```python
from build123d import *

# Parameters (mm, degrees)
CUT_EXTRUDE_1_DEPTH = 4
CUT_EXTRUDE_START   = 31.9
SKETCH_3_R          = 15
SKETCH_3_R_2        = 14.3
CUT_EXTRUDE_2_DEPTH = 1.3


with BuildPart() as part:
    # 草图1 → 旋转1 (revolve)
    with BuildSketch(Plane.XY, mode=Mode.PRIVATE) as revolve_1_sk:
        Polygon((-360, 60), (360, 60), (360, 25), (370, 25), (370, 17.5), (454, 17.5), (454, 0), (-629, 0), (-629, 15), (-583, 15), (-583, 17.5), (-370, 17.5), (-370, 25), (-360, 25), align=None)
    revolve(revolve_1_sk.sketch.rotate(Axis((-629, 0, 0), (1, 0, 0)), 180), axis=Axis((-629, 0, 0), (1, 0, 0)))

    # 草图2 → 切除-拉伸1 (cut)
    with BuildSketch(Plane(origin=(0, 15, 0), x_dir=(1, 0, 0), z_dir=(0, 1, 0))):
        with BuildLine():
            Line((-629, 4), (-593, 4))
            ThreePointArc((-593, 4), (-589, 0), (-593, -4))
            Line((-593, -4), (-629, -4))
            Line((-629, -4), (-629, 4))
        make_face()
    extrude(amount=-CUT_EXTRUDE_1_DEPTH, mode=Mode.SUBTRACT)

    # 草图3 → 切除-拉伸2 (cut)
    with BuildSketch(Plane.ZY.offset(583).offset(CUT_EXTRUDE_START)):
        with Locations(Location((0, 0, 0), (0, 0, 270))):
            Circle(SKETCH_3_R)
        Circle(SKETCH_3_R_2, mode=Mode.SUBTRACT)
    extrude(amount=CUT_EXTRUDE_2_DEPTH, mode=Mode.SUBTRACT)


solid = part.part
```
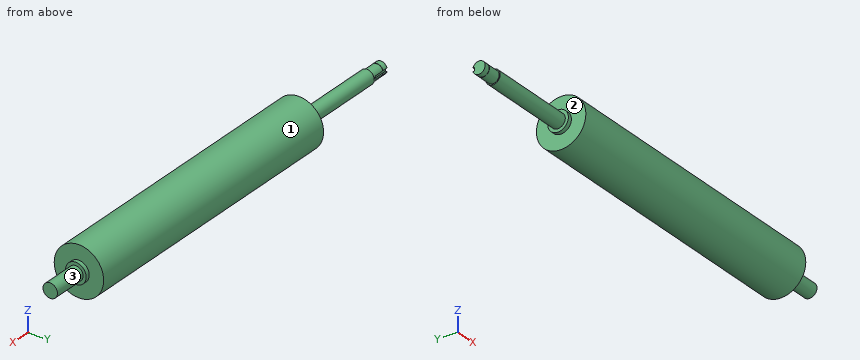
Check sheet for the modelled part. Datum: model origin and axes. Units: mm. Face numbers are marked on the shaded views. A direction names the side the tool comes from. Round coordinates to 2 decimals unless told otherwise and drop trailing zeros. Order: outer loops, then holes, each group sorted by start corner. A loop starts at its lowest first (then second) coordinate and runs counter-clockwise, first axis right, second up.
1) Tool access check on the marked faces 1, 2 and 3. Record the directions out of +Z, -Z, +X, -X, +Y, -Y that give a thin tool (end or side, any length) a straight path to the whole face; none if there is none.
2) Scan lines: line 1 (X direction, y = -10, z = -22.5); line 2 (Y direction, x = -480, z = -0.5); line 3 (Y direction, x = 223.5, z = 2). Record each from-to range of solid material in increasing order.
3) Section check B-B (x = -181). Record the boundary of the cut face in (y, z).
4) Section check D-D (y = 45.5). Record the boundary of the cut face in (x, z), and give its area (3 significant figures).
5) Section check C-C (x = -421). Record the boundary of the cut face in (y, z).
6) Go/stop test with flat-tipped pins: pin 1 Ø5 at (y, z) = (-29, 21.5) entering from +X; pin 2 Ø5 at (y, z) = (38.5, -20) entering from -X; pin 3 Ø8 at (x, y) = (-158.5, 32.5) entering from -Z; pin 4 Ø15 at (y, z) = (9.5, 12) entering from -X. Record where each tip stops, or that it passes through.
Result:
1. face 1: +X, -X
1. face 2: -X
1. face 3: +X
2. line 1: x = -370 to 370
2. line 2: y = -17.49 to 17.49
2. line 3: y = -59.97 to 59.97
3. outline: circle Ø120 at (0, 0)
4. outline: (-360, -39.11) - (360, -39.11) - (360, 39.11) - (-360, 39.11) - close
4. area: 56,300 mm2
5. outline: circle Ø35 at (0, 0)
6. pin 1: stops at x = 360
6. pin 2: stops at x = -360
6. pin 3: stops at z = -52.8
6. pin 4: stops at x = -629
